Source: CAD feature listing. Evaluate the final solid. Frame: model axes, mm. A direction names the side the tool comes from. Give positions to 0.01 mm unless a question says otherwise; leave off trailing zeros. Order: outer loops, then holes, each group sorted by start corner. A loop starts at its lowest first (then second) coordinate and runs counter-clockwise, first axis right, second up.
1) Section B-B, the plane z = -226. Return loops of the section in (x, y), plus the area to 3 significant figures.
2) Section C-C, the plane y = 47. Return loops of the section in (x, z), plus the area to 3 significant figures.
3) Draft query along Y for faces 1 (the face through (-34, 68.5, 6)), 2 (the face through (-34, -72.5, 6)), 3 (the face through (-3, 0, -427)). Return one class per face: released by +Y, released by -Y, zero draft, split by the parting line, or undercut.
4) Material intervals for line 1 (Y direction, x = -17.5, z = 6); line 2 (X direction, y = -25, z = -311); line 3 (Y direction, x = -5.5, z = -110), sorted ascending.
5) Section A-A, the plane x = -17. Return loops of the section in (y, z).
6) First-contact query: P1, Ø4, axis at y = 19.5, z = 331, coming from the -X side. Flat tip, straight axial feed; report the tip coordinate or a pass-through.
7) Access query for faces 4 (the face through (-34, -68.5, 6)), 5 (the face through (-3, 0, 427)). Directions: +Z, -Z, +X, -X, +Y, -Y. A direction counts if a zero-diameter tool reaches every point of the face in a straight line with its end or side. Return the directions, or none.
```python
from build123d import *

# Parameters (mm, degrees)
BOSS_EXTRUDE1_DEPTH = 427


with BuildPart() as part:
    # Sketch1 → Boss-Extrude1 (new, symmetric)
    with BuildSketch(Plane.XY):
        with BuildLine():
            Line((-60, -72.5), (-8, -72.5))
            ThreePointArc((-8, -72.5), (-2.343145751, -70.156854249), (0, -64.5))
            Line((0, -64.5), (0, 64.5))
            ThreePointArc((0, 64.5), (-2.343145751, 70.156854249), (-8, 72.5))
            Line((-8, 72.5), (-60, 72.5))
            Line((-60, 72.5), (-60, 68.5))
            Line((-60, 68.5), (-8, 68.5))
            ThreePointArc((-8, 68.5), (-5.171572875, 67.328427125), (-4, 64.5))
            Line((-4, 64.5), (-4, -64.5))
            ThreePointArc((-4, -64.5), (-5.171572875, -67.328427125), (-8, -68.5))
            Line((-8, -68.5), (-60, -68.5))
            Line((-60, -68.5), (-60, -72.5))
        make_face()
    extrude(amount=BOSS_EXTRUDE1_DEPTH, both=True)


solid = part.part
```
From the geometry:
1. outline: (-60, -72.5) - (-8, -72.5) arc R8 ccw to (0, -64.5) - (0, 64.5) arc R8 ccw to (-8, 72.5) - (-60, 72.5) - (-60, 68.5) - (-8, 68.5) arc R4 cw to (-4, 64.5) - (-4, -64.5) arc R4 cw to (-8, -68.5) - (-60, -68.5) - close
1. area: 1,010 mm2
2. outline: (-4, -427) - (0, -427) - (0, 427) - (-4, 427) - close
2. area: 3,420 mm2
3. face 1: undercut
3. face 2: released by -Y
3. face 3: zero draft
4. line 1: y = -72.5 to -68.5, 68.5 to 72.5
4. line 2: x = -4 to 0
4. line 3: y = -72.1 to -67.62, 67.62 to 72.1
5. outline: (-72.5, -427) - (-68.5, -427) - (-68.5, 427) - (-72.5, 427) - close; (68.5, -427) - (72.5, -427) - (72.5, 427) - (68.5, 427) - close
6. P1: stops at x = -4
7. face 4: +Z, -Z, -X
7. face 5: +Z, +X, -X, +Y, -Y
